Build history of the part. All positions in model axes, mm. Face numbers are marked on the shaded views. A direction names the side the tool comes from. Coordinates: 2 decimals unless noted, no trailing zeros. Write each loop counter-clockwise with the first axis right and the second up, starting at its lowest first coordinate (ties: lowest second). Pieces come first, ordered by that corner, then holes.
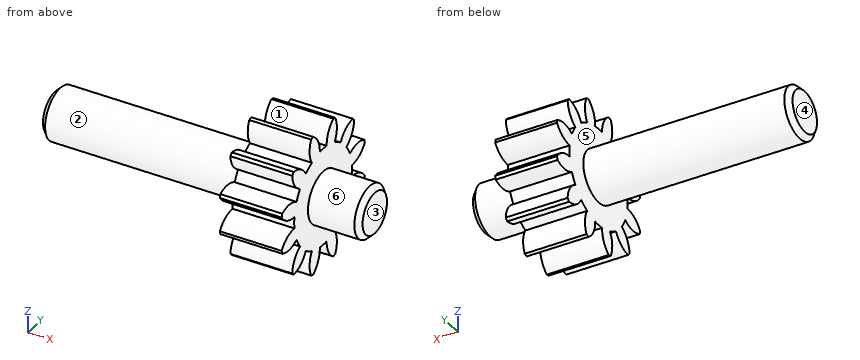
```python
from build123d import *

# Parameters (mm, degrees)
BASPROSKE_W         = 6
BASPROSKE_H         = 7
TOOTHCUT_DEPTH      = 12.575836903
TEETHCUTS_COUNT     = 12
TEETHCUTS_ANGLE     = 330
BORSKE_R            = 0.4
BORE_DEPTH          = 50.0000508
SKETCH1_R           = 2.5
BOSS_EXTRUDE1_DEPTH = 5
BOSS_EXTRUDE2_START = 20
SKETCH2_R           = 2.5
BOSS_EXTRUDE2_DEPTH = 20
CHAMFER1_SIZE       = 0.5


with BuildPart() as part:
    # BasProSke → Base-Revolve (revolve)
    with BuildSketch(Plane(origin=(0, 0, 0), x_dir=(1, 0, 0), z_dir=(0, 1, 0)), mode=Mode.PRIVATE) as base_revolve_sk:
        with Locations((3, 3.5)):
            Rectangle(BASPROSKE_W, BASPROSKE_H)
    revolve(base_revolve_sk.sketch.rotate(Axis((-10, 0, 0), (1, 0, 0)), 180), axis=Axis((-10, 0, 0), (1, 0, 0)))

    # TooCutSke → ToothCut (cut, through all)
    with BuildSketch(Plane(origin=(0, 0, 0), x_dir=(0, 0, -1), z_dir=(1, 0, 0))):
        with BuildLine():
            ThreePointArc((0.562207301, 4.715604304), (0, 4.749), (-0.562207301, 4.715604304))
            ThreePointArc((-0.562207301, 4.715604304), (-0.837528627, 5.917009812), (-1.672850686, 6.823328788))
            ThreePointArc((-1.672850686, 6.823328788), (0, 7.0254), (1.672850686, 6.823328788))
            ThreePointArc((1.672850686, 6.823328788), (0.837528627, 5.917009812), (0.562207301, 4.715604304))
        make_face()
    toothcut = extrude(amount=TOOTHCUT_DEPTH, mode=Mode.SUBTRACT)

    # TeethCuts: ToothCut ×12 about axis
    teethcuts_axis = Axis((-10, 0, 0), (1, 0, 0))
    for i in range(1, TEETHCUTS_COUNT):
        add(toothcut.rotate(teethcuts_axis, i * TEETHCUTS_ANGLE / (TEETHCUTS_COUNT - 1)), mode=Mode.SUBTRACT)

    # BorSke → Bore (cut, symmetric)
    with BuildSketch(Plane(origin=(0, 0, 0), x_dir=(0, 0, -1), z_dir=(1, 0, 0))):
        with Locations(Location((0, 0, 0), (0, 0, 180))):
            Circle(BORSKE_R)
    extrude(amount=BORE_DEPTH, both=True, mode=Mode.SUBTRACT)

    # Sketch1 → Boss-Extrude1 (add)
    with BuildSketch(Plane(origin=(6, 0, 0), x_dir=(0, 0, -1), z_dir=(1, 0, 0))):
        with Locations(Location((0, 0, 0), (0, 0, 180))):
            Circle(SKETCH1_R)
    extrude(amount=BOSS_EXTRUDE1_DEPTH)

    # Sketch2 → Boss-Extrude2 (add)
    with BuildSketch(Plane.ZY.offset(BOSS_EXTRUDE2_START)):
        Circle(SKETCH2_R)
    extrude(amount=-BOSS_EXTRUDE2_DEPTH)

    # Chamfer1
    chamfer1_edges = [part.edges().sort_by_distance(p)[0] for p in [
        (11, 0, -2.5),
        (-20, 0, -2.5),
    ]]
    chamfer(chamfer1_edges, length=CHAMFER1_SIZE)


solid = part.part
```
1. Saw through at C-C on y = 6. List the corners of the cut face in (x, z), plus the area to 3 significant figures.
Computed values:
outline: (0, -2.21) - (6, -2.21) - (6, -0.88) - (0, -0.88) - close; (0, 0.88) - (6, 0.88) - (6, 2.21) - (0, 2.21) - close
area: 15.9 mm2
2. 3-axis set-ups, long thin cutter, end or side, ignore diameter. For the marked faces 4, 5 and 6: which of +Z, -Z, +X, -X, +Y, -Y reach the whole face in a straight line?
Computed values:
face 4: +Z, -Z, -X, +Y, -Y
face 5: -X
face 6: +X
3. Saw through at D-D on x = 9.5. List the corners of the cut face in (y, z), plus the area to 3 significant figures.
Computed values:
outline: circle Ø5 at (0, 0)
area: 19.6 mm2
4. Probe line 1 along Z through (x, y) = (8.5, 1.5); line 2 along X through (y, z) = (2.5, 1); line 3 along Y through (x, z) = (0.5, -5.5). List the from-to ranges inside material, lowest first.
Computed values:
line 1: z = -2 to 2
line 2: x = 0 to 6
line 3: y = -2.23 to -0.67, 0.67 to 2.23
5. Flat gauge pins, fed straight in: pin 1 (3 mm diameter, centred on y = 3.5, z = -0.5, fed in from +X); pin 2 (5 mm diameter, centred on x = -7, z = -2.5, fed in from +Y); pin 3 (5 mm diameter, centred on x = -4, y = 1.5, fed in from -Z). Where does each tip first touch, or does it go through?
Computed values:
pin 1: stops at x = 10.96
pin 2: stops at y = 2.5
pin 3: stops at z = -2.5
6. Saw through at A-A on y = 0. List the corners of the cut face in (x, z).
Computed values:
outline: (-20, -2) - (-19.5, -2.5) - (0, -2.5) - (0, -4.75) - (6, -4.75) - (6, -2.5) - (10.5, -2.5) - (11, -2) - (11, 2) - (10.5, 2.5) - (6, 2.5) - (6, 4.75) - (0, 4.75) - (0, 2.5) - (-19.5, 2.5) - (-20, 2) - close; hole (0, -0.4) - (6, -0.4) - (6, 0.4) - (0, 0.4) - close
7. Mould opens along Y. For the marked faces 1, 2 and 3 say: +Y half, -Y half, draft (parallel to the pull), parting line (faces both ways), or undercut.
Computed values:
face 1: undercut
face 2: parting line
face 3: draft
